Source: three-view drawing plus pictorial views. Frame: mm from the lowest corner of the part. Coordinates: 2 decimals unless noted, no trailing zeros. Loops run counter-clockwise (first coordinate to the right, second up) from the corner with the lowest first, then second, coordinate; pieces in that order, holes last. Notation, with made-up numbers: M -9.75,36.5 L 30.25,36.5 A23 ccw 30.25,55.5 Z; hole C -13,-26.5 d6. An arc over 180 degrees is marked long. Use a Markdown table: item, result. Add a question column.
1. Section B-B on y = 65. Output: boundary loops of the cut face in (x, z).
2. Line query: L1, parallel to Y at x = 287.5, z = 6.75; L2, parallel to X at y = 3.5, z = 6; L3, parallel to X at y = 75.5, z = 1. Output: solid intervals per line, ascending. Write a range as [from, to].
3. Pin query (flat end, axial travel): pin 1 (13 mm diameter, centred on x = 287.5, y = 15, fed in from +Z). Return the tip coordinate at first contact, or that it passes through.
4. Section A-A on x = 12.5. Output: boundary loops of the cut face in (y, z), then the cut area to 3 significant figures.
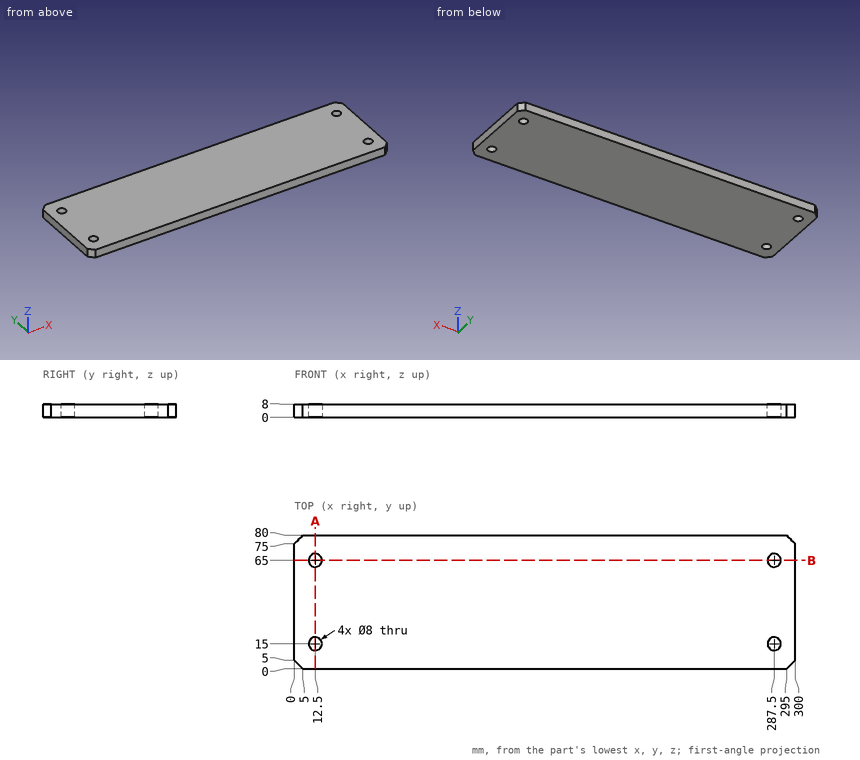
Answers below:
| question | item | result |
|---|---|---|
| 1 | outline | M 0,0 L 8.5,0 L 8.5,8 L 0,8 Z; M 16.5,0 L 283.5,0 L 283.5,8 L 16.5,8 Z; M 291.5,0 L 300,0 L 300,8 L 291.5,8 Z |
| 2 | L1 | y = [0, 11], [19, 61], [69, 80] |
| 2 | L2 | x = [1.5, 298.5] |
| 2 | L3 | x = [0.5, 299.5] |
| 3 | pin 1 | stops at z = 8 |
| 4 | outline | M 0,0 L 11,0 L 11,8 L 0,8 Z; M 19,0 L 61,0 L 61,8 L 19,8 Z; M 69,0 L 80,0 L 80,8 L 69,8 Z |
| 4 | area | 512 mm² |
